from build123d import *

# Parameters (mm, degrees)
BASE_BRACKET_DEPTH          = 6
UPPER_START                 = -28
UPPER_LUG_PLATE_DEPTH       = 12
UPPER_LUG_ROUNDED_END_DEPTH = 12
UPPER_LUG_HOLE_SKETCH_R     = 8
UPPER_LUG_HOLE_16_DEPTH     = 103.46950766
SIDE_LUG_DEPTH              = 12
SIDE_LUG_HOLE_SKETCH_R      = 8
SIDE_LUG_HOLE_16_DEPTH      = 95.093573716
BASE_HOLE_SKETCH_R          = 8
BASE_HOLE_16_DEPTH          = 106.527247666


with BuildPart() as part:
    # Base Profile Sketch → Base Bracket (new, symmetric)
    with BuildSketch(Plane.XY):
        with BuildLine():
            Line((0, 0), (60, 0))
            ThreePointArc((60, 0), (80, 20), (60, 40))
            Line((60, 40), (0, 40))
            Line((0, 40), (0, 0))
        make_face()
    extrude(amount=BASE_BRACKET_DEPTH, both=True)

    # Upper Lug Plate Sketch → Upper Lug Plate (add)
    with BuildSketch(Plane(origin=(0, 40, 0), x_dir=(1, 0, 0), z_dir=(0, 1, 0)).offset(UPPER_START)):
        with BuildLine():
            Line((0, 6), (40, 6))
            Line((40, 6), (40, 30))
            ThreePointArc((40, 30), (20, 50), (0, 30))
            Line((0, 30), (0, 6))
        make_face()
    extrude(amount=-UPPER_LUG_PLATE_DEPTH)

    # Upper Lug End Sketch → Upper Lug Rounded End (add)
    with BuildSketch(Plane(origin=(0, 40, 0), x_dir=(1, 0, 0), z_dir=(0, 1, 0))):
        with BuildLine():
            Line((40.095269472, 30), (40, 30))
            Line((40, 30), (40, 6))
            Line((40, 6), (0, 6))
            Line((0, 6), (0, 30))
            Line((0, 30), (0.095269472, 30))
            ThreePointArc((0.095269472, 30), (20.095269472, 50), (40.095269472, 30))
        make_face()
    extrude(amount=-UPPER_LUG_ROUNDED_END_DEPTH)

    # Upper Lug Hole Sketch → Upper Lug Hole Ø16 (cut, through all)
    with BuildSketch(Plane(origin=(0, 40, 0), x_dir=(1, 0, 0), z_dir=(0, 1, 0))):
        with Locations(Location((20.095269472, 30, 0), (0, 0, 270))):
            Circle(UPPER_LUG_HOLE_SKETCH_R)
    extrude(amount=-UPPER_LUG_HOLE_16_DEPTH, mode=Mode.SUBTRACT)

    # Side Lug Sketch → Side Lug (add)
    with BuildSketch(Plane.ZY):
        with BuildLine():
            Line((6, 40), (31.279631577, 40))
            ThreePointArc((31.279631577, 40), (51.279631577, 20), (31.279631577, 0))
            Line((31.279631577, 0), (6, 0))
            Line((6, 0), (6, 40))
        make_face()
    extrude(amount=-SIDE_LUG_DEPTH)

    # Side Lug Hole Sketch → Side Lug Hole Ø16 (cut, through all)
    with BuildSketch(Plane(origin=(12, 0, 0), x_dir=(0, 0, -1), z_dir=(1, 0, 0))):
        with Locations((-31.279631577, 20)):
            Circle(SIDE_LUG_HOLE_SKETCH_R)
    extrude(amount=-SIDE_LUG_HOLE_16_DEPTH, mode=Mode.SUBTRACT)

    # Base Hole Sketch → Base Hole Ø16 (cut, through all)
    with BuildSketch(Plane.XY.offset(6)):
        with Locations((60, 20)):
            Circle(BASE_HOLE_SKETCH_R)
    extrude(amount=-BASE_HOLE_16_DEPTH, mode=Mode.SUBTRACT)


solid = part.part
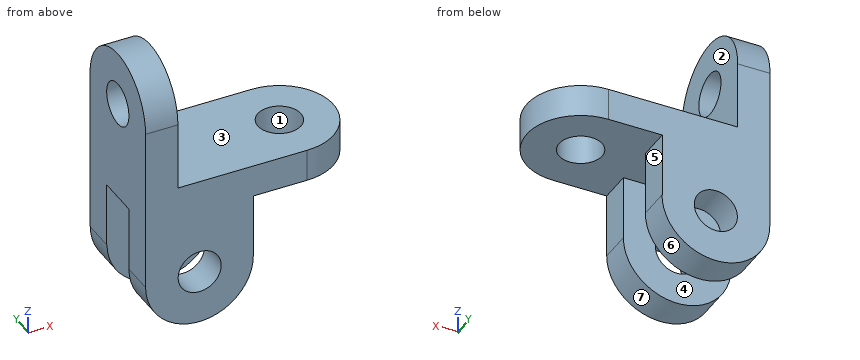
Check sheet for the modelled part. Datum: model origin and axes. Units: mm. Face numbers are marked on the shaded views. A direction names the side the tool comes from. Round coordinates to 2 decimals unless told otherwise and drop trailing zeros. Order: outer loops, then holes, each group sorted by start corner. A loop starts at its lowest first (then second) coordinate and runs counter-clockwise, first axis right, second up.
(1) Access from +Z, -Z, +X, -X, +Y, -Y to the whole of each face (thin tool, end or side, straight path). Record for the marked faces 4, 5, 6 and 7.
(2) Draft check along X on the marked faces 1, 2 and 3. Enter one of: pulls with the +X half, pulls with the -X half, needs draft (parallel to the pull), parting line crosses it, or undercut.
(3) Cross-section at A-A, the plane z = -11.5. Enter the section's corners in (x, y).
(4) Go/stop test with flat-tipped pins: P1, Ø8, axis at x = 18.5, z = 34.5, coming from the -Y side; P2, Ø6, axis at y = 33.5, z = -21.5, coming from the +X side; P3, Ø12, axis at x = 40, y = 13, coming from the +Z side; P4, Ø10, axis at x = 16.5, y = 6, coming from the +Z side. Record where each tip stops, or that it passes through.
(5) Scan lines: probe 1 along X at (y, z) = (2, -30); probe 2 along Y at (x, z) = (15, -11.5); probe 3 along Z at (x, y) = (44, 28). Record each from-to range of solid material in increasing order.
(6) Cross-section at C-C, the plane y = 25.5. Enter the section's corners in (x, z).
(7) Cross-section at D-D, the plane x = 18.5. Enter the section's corners in (y, z), and give its area (3 significant figures).
Check sheet entries:
1. face 4: -Z, +X, -X
1. face 5: +X, +Y, -Y
1. face 6: -Z, +Y
1. face 7: -Z, -Y
2. face 1: undercut
2. face 2: pulls with the +X half
2. face 3: needs draft
3. outline: (0, 0) - (40, 0) - (40, 12) - (0, 12) - close; (0, 28) - (40, 28) - (40, 40) - (0, 40) - close
4. P1: passes through
4. P2: stops at x = 40
4. P3: stops at z = 6
4. P4: stops at z = 47.41
5. probe 1: x = 0 to 12.1, 28.1 to 40
5. probe 2: y = 0 to 12, 28 to 40
5. probe 3: z = -6 to 6
6. outline: (0, -6) - (54.19, -6) - (54.19, 6) - (12, 6) - (12, 25.47) - (0, 25.47) - close; (0, 37.09) - (12, 37.09) - (12, 50.51) - (0, 50.51) - close; (65.81, -6) - (79.23, -6) - (79.23, 6) - (65.81, 6) - close
7. outline: (0, -49.94) - (12, -49.94) - (12, -37.84) - (0, -37.84) - close; (0, -22.16) - (12, -22.16) - (12, -6) - (28, -6) - (28, -22.16) - (40, -22.16) - (40, 6) - (0, 6) - close; (28, -49.94) - (40, -49.94) - (40, -37.84) - (28, -37.84) - close
7. area: 1,160 mm2
